Model file for the job. Use its own axes, mm. A direction names the side the tool comes from. Coordinates: 2 decimals unless noted, no trailing zeros. Write each loop counter-clockwise with the first axis right and the second up, starting at its lowest first coordinate (ties: lowest second). Pieces come first, ordered by that corner, then holes. Notation, with made-up numbers: M 11,76 L 17,76 A34 cw 17,109 Z; hole C 24.25,56.5 d9. An arc over 180 degrees is marked long. One line per question, with ' | ' between items. Start each with the question number.
(1) Cut at B-B (y = 0). Write the cut outline in (x, z), plus the area to 3 significant figures.
(2) Cut at C-C (x = 3). Write the cut outline in (y, z), plus the area to 3 significant figures.
(3) Wall check: probe 1 along X at (y, z) = (9.2, -5); probe 2 along X at (y, z) = (-5, -4); probe 3 along Y at (x, z) = (20.5, -3.25). Give the ranges that are in metal, low to high.
(4) Flat gauge pins, fed straight in: pin 1 Ø2 at (x, z) = (12, -4) entering from -Y; pin 2 Ø1.5 at (y, z) = (-4, -5) entering from +X; pin 3 Ø1.5 at (x, y) = (22, -6.5) entering from -Z. Where does each tip first touch, or does it go through?
(5) Cut at A-A (z = -5.75). Write the cut outline in (x, y).
(6) Tool access for faces 1 (the face through (12.28, 4.24, -6.2)), 2 (the face through (16.06, -11.51, -6.77)), 3 (the face through (13, 0, 0)), 4 (the face through (1.718, 0.175, -1.025)), 5 (the face through (9.382, 10.035, -3.656)): list every direction of +Z, -Z, +X, -X, +Y, -Y with a clear straight run to the whole face (end or side of a thin tool).
(7) Two-plate mould, pull along Y, no slides. Class faces 6 (the face through (13, -10.5, -5)), 7 (the face through (19, 7.5, -3)), 8 (the face through (22.823, 0.175, -6.451)), 9 (the face through (12.28, -5.76, -6.2)): +Y half, -Y half, draft (parallel to the pull), parting line (faces both ways), or undercut.
from build123d import *

# Parameters (mm, degrees)
BOSS_EXTRUDE1_DEPTH        = 12.5
SKETCH2_R                  = 2.5
CUT_EXTRUDE1_DEPTH         = 5
M3_TAPPED_HOLE1_D          = 2.5
M3_TAPPED_HOLE1_DEPTH      = 7.5
M3_TAPPED_HOLE1_TIP        = 0.751075774
F_3_2_3_2_DIAMETER_HOLE1_D = 3.2
SKETCH8_R                  = 3.3
CUT_EXTRUDE2_DEPTH         = 2


with BuildPart() as part:
    # Sketch1 → Boss-Extrude1 (new, symmetric)
    with BuildSketch(Plane(origin=(0, 0, 0), x_dir=(1, 0, 0), z_dir=(0, 1, 0))):
        with BuildLine():
            Line((3.464101615, 0), (23.082903769, 0))
            ThreePointArc((23.082903769, 0), (24.814954576, 1), (24.814954576, 3))
            Line((24.814954576, 3), (20.773502692, 10))
            Line((20.773502692, 10), (5.773502692, 10))
            Line((5.773502692, 10), (1.732050808, 3))
            ThreePointArc((1.732050808, 3), (1.732050808, 1), (3.464101615, 0))
        make_face()
    extrude(amount=BOSS_EXTRUDE1_DEPTH, both=True)

    # Sketch2 → Cut-Extrude1 (cut)
    with BuildSketch(Plane(origin=(0, 12.5, 0), x_dir=(1, 0, 0), z_dir=(0, 1, 0))):
        with Locations(Location((7.273502692, 5, 0), (0, 0, 270))):
            Circle(SKETCH2_R)
        with Locations(Location((19.273502692, 5, 0), (0, 0, 270))):
            Circle(SKETCH2_R)
    extrude(amount=-CUT_EXTRUDE1_DEPTH, mode=Mode.SUBTRACT)

    # M3 Tapped Hole1
    with Locations(Plane(origin=(0, 0, -10), x_dir=(-1, 0, 0), z_dir=(0, 0, -1))):
        with Locations((-13.273502692, -5), (-13.273502692, 5)):
            Hole(M3_TAPPED_HOLE1_D / 2, depth=M3_TAPPED_HOLE1_DEPTH)
            with Locations((0, 0, -(M3_TAPPED_HOLE1_DEPTH + M3_TAPPED_HOLE1_TIP / 2))):  # 118° drill point
                Cone(0, M3_TAPPED_HOLE1_D / 2, M3_TAPPED_HOLE1_TIP, mode=Mode.SUBTRACT)

    # Ø3.2 (3.2) Diameter Hole1 (through all)
    with Locations(Plane(origin=(0, 7.5, 0), x_dir=(-1, 0, 0), z_dir=(0, 1, 0))):
        with Locations((-19.273502692, -5), (-7.273502692, -5)):
            Hole(F_3_2_3_2_DIAMETER_HOLE1_D / 2)

    # Sketch8 → Cut-Extrude2 (cut)
    with BuildSketch(Plane.XZ.offset(12.5)):
        with Locations(Location((13.273502692, -5, 0), (0, 0, 270))):
            Circle(SKETCH8_R)
    extrude(amount=-CUT_EXTRUDE2_DEPTH, mode=Mode.SUBTRACT)


solid = part.part
Filled in:
1) outline: M 1.73,-3 L 5.77,-10 L 20.77,-10 L 24.81,-3 A2 ccw 23.08,0 L 3.46,0 A2 ccw Z; hole C 7.27,-5 d3.2; hole C 19.27,-5 d3.2 | area: 186 mm²
2) outline: M -12.5,-5.2 L 12.5,-5.2 L 12.5,-0.05 L -12.5,-0.05 Z | area: 129 mm²
3) probe 1: 2.89 to 4.77, 9.77 to 16.77, 21.77 to 23.66 | probe 2: 2.31 to 6.02, 8.52 to 12.02, 14.52 to 18.02, 20.52 to 24.24 | probe 3: -12.5 to 7.5
4) pin 1: y = -10.5 | pin 2: x = 24.09 | pin 3: z = -9.17
5) outline: M 3.32,-12.5 L 5.86,-12.5 L 5.86,7.5 L 4.89,7.5 L 4.89,12.5 L 3.32,12.5 Z; M 8.69,-12.5 L 10.06,-12.5 L 10.06,-10.5 L 16.49,-10.5 L 16.49,-12.5 L 17.86,-12.5 L 17.86,7.5 L 16.89,7.5 L 16.89,12.5 L 9.66,12.5 L 9.66,7.5 L 8.69,7.5 Z; M 20.69,-12.5 L 23.23,-12.5 L 23.23,12.5 L 21.66,12.5 L 21.66,7.5 L 20.69,7.5 Z; hole C 13.27,-5 d2.5; hole C 13.27,5 d2.5
6) face 1: -Z | face 2: -Y | face 3: +Z, +X, -X, +Y, -Y | face 4: -X, +Y, -Y | face 5: +Y
7) face 6: -Y half | face 7: +Y half | face 8: draft | face 9: undercut
